Source: CAD feature listing. Evaluate the final solid. Frame: model axes, mm. Face numbers are marked on the shaded views. A direction names the side the tool comes from. Give positions to 0.01 mm unless a question says otherwise; leave off trailing zeros. Order: outer loops, then holes, each group sorted by start corner. A loop starts at its lowest first (then second) coordinate and runs counter-clockwise, first axis right, second up. Notation, with made-up numbers: M 66.5,40 L 102.5,40 A22 cw 102.5,50 Z; hole C 77.25,25 d7. An arc over 180 degrees is marked long. Answer in a Markdown table with one row per item. Add a question column.
(1) Set-up query: the marked faces 1 and 2. Return all of +Z, -Z, +X, -X, +Y, -Y with unobstructed straight access to the full face (end or side cutting, diameter ignored); none if empty.
(2) Pin query (flat end, axial travel): P1, Ø8, axis at x = 153, z = -7.5, coming from the -Y side; P2, Ø1, axis at x = 39.5, z = 5, coming from the +Y side; P3, Ø2, axis at x = 46.5, z = -5, coming from the +Y side. Return the tip coordinate at first contact, or that it passes through.
(3) Section query A-A, the plane y = 0. Return loops of the section in (x, z).
(4) Material intervals for line 1 along X through (y, z) = (-5.5, 0); line 2 along X through (y, z) = (-4.5, 3.25); line 3 along X through (y, z) = (-6.75, 6), sorted ascending.
(5) Section query B-B, the plane x = 173. Return loops of the section in (y, z), plus the area to 3 significant figures.
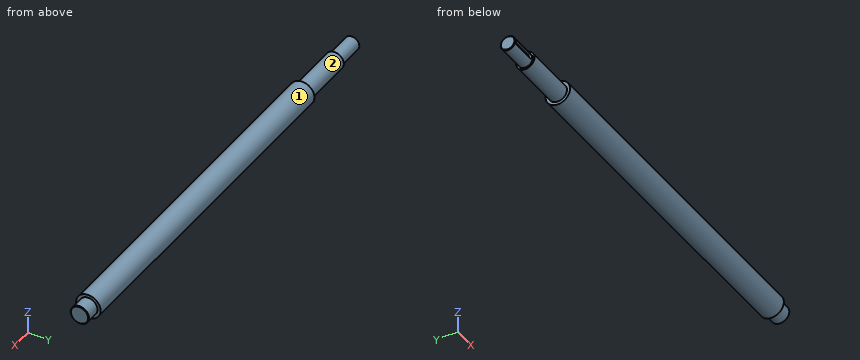
from build123d import *

# Parameters (mm, degrees)
CUT_EXTRUDE_1_DEPTH = 2.2
CHAMFER_1_SIZE      = 0.5


with BuildPart() as part:
    # 草图1 → 旋转1 (revolve)
    with BuildSketch(Plane(origin=(0, 0, 0), x_dir=(1, 0, 0), z_dir=(0, 1, 0)), mode=Mode.PRIVATE) as revolve_1_sk:
        Polygon((0, 0), (0, 6), (24, 6), (24, 7.5), (68, 7.5), (68, 10), (358, 10), (358, 7.5), (370, 7.5), (370, 0), align=None)
    revolve(revolve_1_sk.sketch.rotate(Axis((0, 0, 0), (1, 0, 0)), 180), axis=Axis((0, 0, 0), (1, 0, 0)))

    # 草图2 → 切除-拉伸1 (cut)
    with BuildSketch(Plane(origin=(0, -6, 0), x_dir=(-1, 0, 0), z_dir=(0, -1, 0))):
        with BuildLine():
            Line((-21, 2), (-3, 2))
            ThreePointArc((-3, 2), (-1, 0), (-3, -2))
            Line((-3, -2), (-21, -2))
            ThreePointArc((-21, -2), (-23, 0), (-21, 2))
        make_face()
    extrude(amount=-CUT_EXTRUDE_1_DEPTH, mode=Mode.SUBTRACT)

    # 倒角1
    chamfer_1_edges = [part.edges().sort_by_distance(p)[0] for p in [
        (0, 0, -6),
        (370, 0, -7.5),
    ]]
    chamfer(chamfer_1_edges, length=CHAMFER_1_SIZE)


solid = part.part
Values follow:
| question | item | result |
|---|---|---|
| 1 | face 1 | +X, -X |
| 1 | face 2 | -X |
| 2 | P1 | stops at y = -9.37 |
| 2 | P2 | stops at y = 6 |
| 2 | P3 | stops at y = 6.34 |
| 3 | outline | M 0,-5.5 L 0.5,-6 L 24,-6 L 24,-7.5 L 68,-7.5 L 68,-10 L 358,-10 L 358,-7.5 L 369.5,-7.5 L 370,-7 L 370,7 L 369.5,7.5 L 358,7.5 L 358,10 L 68,10 L 68,7.5 L 24,7.5 L 24,6 L 0.5,6 L 0,5.5 Z |
| 4 | line 1 | x = 0 to 1, 23 to 370 |
| 4 | line 2 | x = 0.05 to 370 |
| 4 | line 3 | x = 68 to 358 |
| 5 | outline | C 0,0 d20 |
| 5 | area | 314 mm² |
